from build123d import *

# Parameters (mm, degrees)
SKETCH_1_W          = 62
SKETCH_1_H          = 66
EXTRUDE_1_DEPTH     = 6
SKETCH_3_W          = 58.1
SKETCH_3_H          = 113.69115984
CUT_EXTRUDE_1_DEPTH = 2
HOLE_WIZARD_M4_1_D  = 3.3
HOLE_WIZARD_M4_2_D  = 3.3
SKETCH_14_W         = 98
SKETCH_14_H         = 12
EXTRUDE_3_DEPTH     = 10
CUT_EXTRUDE_2_DEPTH = 75.652528423
SKETCH_16_W         = 58.1
SKETCH_16_H         = 41.285826149
CUT_EXTRUDE_3_DEPTH = 2
SKETCH_17_W         = 126.235416792
SKETCH_17_H         = 53.479043567
CUT_EXTRUDE_4_DEPTH = 2
CHAMFER_1_SIZE      = 1
CHAMFER_2_SIZE      = 1


with BuildPart() as part:
    # 草图1 → 凸台-拉伸1 (new, symmetric)
    with BuildSketch(Plane.XY):
        Rectangle(SKETCH_1_W, SKETCH_1_H)
    extrude(amount=EXTRUDE_1_DEPTH, both=True)

    # 草图3 → 切除-拉伸1 (cut)
    with BuildSketch(Plane.XY.offset(6)):
        Rectangle(SKETCH_3_W, SKETCH_3_H)
    extrude(amount=-CUT_EXTRUDE_1_DEPTH, mode=Mode.SUBTRACT)

    # M4 螺纹孔1 (through all)
    with Locations(Plane.XY.offset(4)):
        with Locations((-11.5, 28), (11.5, 28), (-11.5, 8), (11.5, 8)):
            Hole(HOLE_WIZARD_M4_1_D / 2)

    # M4 螺纹孔2 (through all)
    with Locations(Plane(origin=(0, 0, -6), x_dir=(-1, 0, 0), z_dir=(0, 0, -1))):
        with Locations((-16, 22), (16, 22)):
            Hole(HOLE_WIZARD_M4_2_D / 2)

    # 草图14 → 凸台-拉伸3 (add)
    with BuildSketch(Plane.XZ.offset(33)):
        Rectangle(SKETCH_14_W, SKETCH_14_H)
    extrude(amount=-EXTRUDE_3_DEPTH)

    # 草图15 → 切除-拉伸2 (cut, through all)
    with BuildSketch(Plane(origin=(0, -23, 0), x_dir=(1, 0, 0), z_dir=(0, 1, 0))):
        with BuildLine():
            Line((-43, 2.7), (-37, 2.7))
            ThreePointArc((-37, 2.7), (-34.3, 0), (-37, -2.7))
            Line((-37, -2.7), (-43, -2.7))
            ThreePointArc((-43, -2.7), (-45.7, 0), (-43, 2.7))
        make_face()
    cut_extrude_2 = extrude(amount=-CUT_EXTRUDE_2_DEPTH, mode=Mode.SUBTRACT)

    # 镜向1: 切除-拉伸2 across plane
    add(cut_extrude_2.mirror(Plane(origin=(0, 0, 0), x_dir=(0, 0, 1), z_dir=(1, 0, 0))), mode=Mode.SUBTRACT)

    # 草图16 → 切除-拉伸3 (cut)
    with BuildSketch(Plane.XY.offset(6)):
        with Locations((0, -39.137864824)):
            Rectangle(SKETCH_16_W, SKETCH_16_H)
    extrude(amount=-CUT_EXTRUDE_3_DEPTH, mode=Mode.SUBTRACT)

    # 草图17 → 切除-拉伸4 (cut)
    with BuildSketch(Plane(origin=(0, 0, -6), x_dir=(-1, 0, 0), z_dir=(0, 0, -1))):
        with Locations((-8.783621981, 43.739521784)):
            Rectangle(SKETCH_17_W, SKETCH_17_H)
    extrude(amount=-CUT_EXTRUDE_4_DEPTH, mode=Mode.SUBTRACT)

    # 倒角1
    chamfer_1_edges = [part.edges().sort_by_distance(p)[0] for p in [
        (49, -28, -6),
        (-49, -28, 6),
        (49, -28, 6),
        (-49, -28, -6),
    ]]
    chamfer(chamfer_1_edges, length=CHAMFER_1_SIZE)

    # 倒角2
    chamfer_2_edges = [part.edges().sort_by_distance(p)[0] for p in [
        (-31, 33, 1),
        (31, 33, 1),
    ]]
    chamfer(chamfer_2_edges, length=CHAMFER_2_SIZE)


solid = part.part
Build history of the part. All positions in model axes, mm. A direction names the side the tool comes from. Round coordinates to 2 decimals unless told otherwise and drop trailing zeros. Write each loop counter-clockwise with the first axis right and the second up, starting at its lowest first coordinate (ties: lowest second). Pieces come first, ordered by that corner, then holes. Notation, with made-up numbers: M 69,-17.5 L 90,-17.5 A9 ccw 90,-12.5 Z; hole C 58.25,6.5 d6. An arc over 180 degrees is marked long. Answer in a Markdown table with one row per item.
1. Which spindle directions (+Z, -Z, +X, -X, +Y, -Y) get a long thin tool onto all of the face, cutting with end or side? Do faces 1 (the face through (-29.05, 0, 5)), 2 (the face through (-12.39, 29.39, -0.06)), 3 (the face through (40, -28, 2.7)), 4 (the face through (0, 25, -4)), 5 (the face through (-40, -23, 3)). Say none if no direction does.
Geometry check:
| item | result |
|---|---|
| face 1 | +Z, +Y, -Y |
| face 2 | +Z, -Z |
| face 3 | +Y, -Y |
| face 4 | -Z, +X, -X, +Y |
| face 5 | +Z, -Z, -X, +Y |
2. Saw through at D-D (y = -16.5). List the corners of the cut face in (x, z).
Geometry check:
| item | result |
|---|---|
| outline | M -31,-6 L 31,-6 L 31,6 L 29.05,6 L 29.05,4 L -29.05,4 L -29.05,6 L -31,6 Z |
3. Mould opens along X. For faces 6 (the face through (45.7, -27.9, 0.1)), 7 (the face through (-49, -28, 0)), 8 (the face through (0, 17, -5)) say: +X half, -X half, draft (parallel to the pull), parting line (faces both ways), or undercut.
Geometry check:
| item | result |
|---|---|
| face 6 | undercut |
| face 7 | -X half |
| face 8 | draft |
4. Saw through at B-B (y = 8). List the corners of the cut face in (x, z), and give its area (3 significant figures).
Geometry check:
| item | result |
|---|---|
| outline | M -31,-6 L -13.15,-6 L -13.15,4 L -29.05,4 L -29.05,6 L -31,6 Z; M -9.85,-6 L 9.85,-6 L 9.85,4 L -9.85,4 Z; M 13.15,-6 L 31,-6 L 31,6 L 29.05,6 L 29.05,4 L 13.15,4 Z |
| area | 562 mm2 |
5. Saw through at C-C (z = 1). State how many separate pieces and enclosed holes the cut face has, and give its area (3 significant figures).
Geometry check:
| item | result |
|---|---|
| separate pieces | 3 |
| enclosed holes | 6 |
| area | 4,180 mm2 |
6. Saw through at A-A (x = -16). List the corners of the cut face in (y, z).
Geometry check:
| item | result |
|---|---|
| outline | M -33,-6 L 17,-6 L 17,-4 L 20.35,-4 L 20.35,4 L -33,4 Z; M 23.65,-4 L 33,-4 L 33,4 L 23.65,4 Z |
7. Flat gauge pins, fed straight in: P1, Ø3, axis at y = -17.5, z = -4, coming from the +X side; P2, Ø10, axis at x = -33, y = -18, coming from the +Z side; P3, Ø5.5, axis at x = 16, y = 22, coming from the -Z side; P4, Ø1.6, axis at x = 5.5, z = -5.5, coming from the +Y side. Where does each tip first touch, or does it go through?
Geometry check:
| item | result |
|---|---|
| P1 | x = 31 |
| P2 | z = 6 |
| P3 | z = -4 |
| P4 | y = 17 |
8. Probe L1, parallel to Y at x = -11.5, z = -2.5; L2, parallel to X at y = 25.5, z = 5; L3, parallel to Z at x = -16, y = 0. List the from-to ranges inside material, lowest first. Write a range as [from, to].
Geometry check:
| item | result |
|---|---|
| L1 | [-33, 6.35], [9.65, 26.35], [29.65, 33] |
| L2 | [-31, -29.05], [29.05, 31] |
| L3 | [-6, 4] |
